from build123d import *

# Parameters (mm, degrees)
SKETCH1_W                                            = 120
SKETCH1_H                                            = 32
BOSS_EXTRUDE1_DEPTH                                  = 15
SKETCH2_W                                            = 120
SKETCH2_H                                            = 15
CUT_EXTRUDE1_DEPTH                                   = 2
F_8_0MM_BLIND_HOLE_1_D                               = 8
F_8_0MM_BLIND_HOLE_1_DEPTH                           = 6
F_8_0MM_BLIND_HOLE_1_TIP                             = 2.403442476
M8_CLEARANCE_HOLE1_D                                 = 9
CHAMFER1_SIZE                                        = 2
CBORE_FOR_M5_HEXAGON_SOCKET_HEAD_CAP_SCR_D           = 5.5
CBORE_FOR_M5_HEXAGON_SOCKET_HEAD_CAP_SCR_CBORE_D     = 10
CBORE_FOR_M5_HEXAGON_SOCKET_HEAD_CAP_SCR_CBORE_DEPTH = 5.7
CBORE_FOR_M6_HEXAGON_SOCKET_HEAD_CAP_SCR_D           = 6.6
CBORE_FOR_M6_HEXAGON_SOCKET_HEAD_CAP_SCR_CBORE_D     = 11
CBORE_FOR_M6_HEXAGON_SOCKET_HEAD_CAP_SCR_CBORE_DEPTH = 6.8
F_5_0MM_BLIND_HOLE_1_D                               = 5


with BuildPart() as part:
    # Sketch1 → Boss-Extrude1 (new body)
    with BuildSketch(Plane(origin=(0, 0, 0), x_dir=(0, 0, -1), z_dir=(1, 0, 0))):
        Rectangle(SKETCH1_W, SKETCH1_H)
    extrude(amount=BOSS_EXTRUDE1_DEPTH)

    # Sketch2 → Cut-Extrude1 (cut)
    with BuildSketch(Plane(origin=(15, 0, 0), x_dir=(0, 0, -1), z_dir=(1, 0, 0))):
        with Locations((0, -8.5)):
            Rectangle(SKETCH2_W, SKETCH2_H)
    extrude(amount=-CUT_EXTRUDE1_DEPTH, mode=Mode.SUBTRACT)

    # Ø8.0mm blind hole 1
    with Locations(Plane.ZY):
        with Locations((35, 8.5), (-35, 8.5)):
            Hole(F_8_0MM_BLIND_HOLE_1_D / 2, depth=F_8_0MM_BLIND_HOLE_1_DEPTH)
            with Locations((0, 0, -(F_8_0MM_BLIND_HOLE_1_DEPTH + F_8_0MM_BLIND_HOLE_1_TIP / 2))):  # 118° drill point
                Cone(0, F_8_0MM_BLIND_HOLE_1_D / 2, F_8_0MM_BLIND_HOLE_1_TIP, mode=Mode.SUBTRACT)

    # M8 Clearance Hole1 (through all)
    with Locations(Plane(origin=(15, 0, 0), x_dir=(0, 0, -1), z_dir=(1, 0, 0))):
        with Locations((-20, 8.5)):
            Hole(M8_CLEARANCE_HOLE1_D / 2)

    # Chamfer1
    chamfer1_edges = [part.edges().sort_by_distance(p)[0] for p in [
        (6.5, -16, -60),
        (6.5, -16, 60),
        (7.5, 16, 60),
        (7.5, 16, -60),
    ]]
    chamfer(chamfer1_edges, length=CHAMFER1_SIZE)

    # CBORE for M5 Hexagon socket head cap screws1 (through all)
    with Locations(Plane(origin=(15, 0, 0), x_dir=(0, 0, -1), z_dir=(1, 0, 0))):
        with Locations((-35, 8.5), (35, 8.5)):
            CounterBoreHole(CBORE_FOR_M5_HEXAGON_SOCKET_HEAD_CAP_SCR_D / 2, CBORE_FOR_M5_HEXAGON_SOCKET_HEAD_CAP_SCR_CBORE_D / 2, CBORE_FOR_M5_HEXAGON_SOCKET_HEAD_CAP_SCR_CBORE_DEPTH)

    # CBORE for M6 Hexagon socket head cap screws1 (through all)
    with Locations(Plane.ZY):
        with Locations((-27.5, -8.5), (52.5, -8.5)):
            CounterBoreHole(CBORE_FOR_M6_HEXAGON_SOCKET_HEAD_CAP_SCR_D / 2, CBORE_FOR_M6_HEXAGON_SOCKET_HEAD_CAP_SCR_CBORE_D / 2, CBORE_FOR_M6_HEXAGON_SOCKET_HEAD_CAP_SCR_CBORE_DEPTH)

    # Ø5.0mm blind hole 1 (through all)
    with Locations(Plane.ZY):
        with Locations((22.5, -8.5)):
            Hole(F_5_0MM_BLIND_HOLE_1_D / 2)


solid = part.part
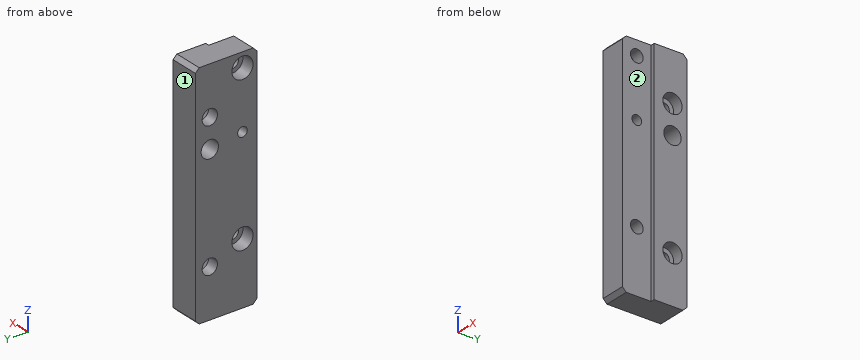
Here's how the part is built. I have some questions about the finished solid (model axes, mm). Face numbers are marked on the shaded views. A direction names the side the tool comes from. Round coordinates to 2 decimals unless told otherwise and drop trailing zeros. Order: outer loops, then holes, each group sorted by start corner. A loop starts at its lowest first (then second) coordinate and runs counter-clockwise, first axis right, second up. Notation, with made-up numbers: (-8, 50.5) -> (1, 50.5) arc R29 cw to (1, 82.5) -> close; hole circle Ø3 at (64, 3). An arc over 180 degrees is marked (long way). Return JSON: item names as keys, results as strings.
Q1. If we section it at A-A on y = 8.5: Give the number of separate pieces and of enclosed holes in the cut face, plus the area to 3 significant figures.
Filled sheet:
{"separate pieces": "4", "enclosed holes": "0", "area": "1,420 mm^2"}
Q2. If we section it at B-B on x = 4.5: List the corners of the cut face in (y, z) for me.
Filled sheet:
{"outline": "(-16, -58) -> (-14, -60) -> (14, -60) -> (16, -58) -> (16, 58) -> (14, 60) -> (-14, 60) -> (-16, 58) -> close; hole circle Ø11 at (-8.5, -27.5); hole circle Ø11 at (-8.5, 52.5); hole circle Ø5 at (-8.5, 22.5); hole circle Ø9 at (8.5, 20); hole circle Ø8 at (8.5, -35); hole circle Ø8 at (8.5, 35)"}
Q3. I need wall thicknesses on line 1 along Y through (x, z) = (2.15, -35); line 2 along Z through (x, y) = (13.25, 11.5); line 3 along Y through (x, z) = (4, -27.5). Which ranges of each line are inside material? Lowest first, please. Write a range as from..to.
Filled sheet:
{"line 1": "y = -16..4.5, 12.5..16", "line 2": "z = -60..-39, -31..16.65, 23.35..31, 39..60", "line 3": "y = -16..-14, -3..16"}
Q4. If we section it at C-C on z = -27.5: List the corners of the cut face in (x, y) for me.
Filled sheet:
{"outline": "(0, -16) -> (13, -16) -> (13, -11.8) -> (6.8, -11.8) -> (6.8, -14) -> (0, -14) -> close; (0, -3) -> (6.8, -3) -> (6.8, -5.2) -> (13, -5.2) -> (13, -1) -> (15, -1) -> (15, 16) -> (0, 16) -> close"}
Q5. For pin 1 Ø7 at (y, z) = (8.5, -35) entering from -X; pin 2 Ø5 at (y, z) = (9.5, 36.5) entering from +X; pin 3 Ø0.6 at (x, z) = (13.5, 3) entering from -Y, each with a flat end and sliding along its axis, tell me the tip position at first contact or that it passes through.
Filled sheet:
{"pin 1": "stops at x = 6.3", "pin 2": "stops at x = 9.3", "pin 3": "stops at y = -1"}
Q6. Which directions (+Z, -Z, +X, -X, +Y, -Y) give clear straight access to the entire face, cutting with the end or side of a thin tool? Please do the marked faces 1 and 2.
Filled sheet:
{"face 1": "+Z, -Z, +X, -X, +Y", "face 2": "+Z, -Z, +X, -Y"}
Q7. If we section it at D-D on z = 35: List the corners of the cut face in (x, y) for me, plus the area to 3 significant figures.
Filled sheet:
{"outline": "(0, -16) -> (13, -16) -> (13, -1) -> (15, -1) -> (15, 3.5) -> (9.3, 3.5) -> (9.3, 5.75) -> (6.75, 5.75) -> (6, 4.5) -> (0, 4.5) -> close; (0, 12.5) -> (6, 12.5) -> (6.75, 11.25) -> (9.3, 11.25) -> (9.3, 13.5) -> (15, 13.5) -> (15, 16) -> (0, 16) -> close", "area": "326 mm^2"}
